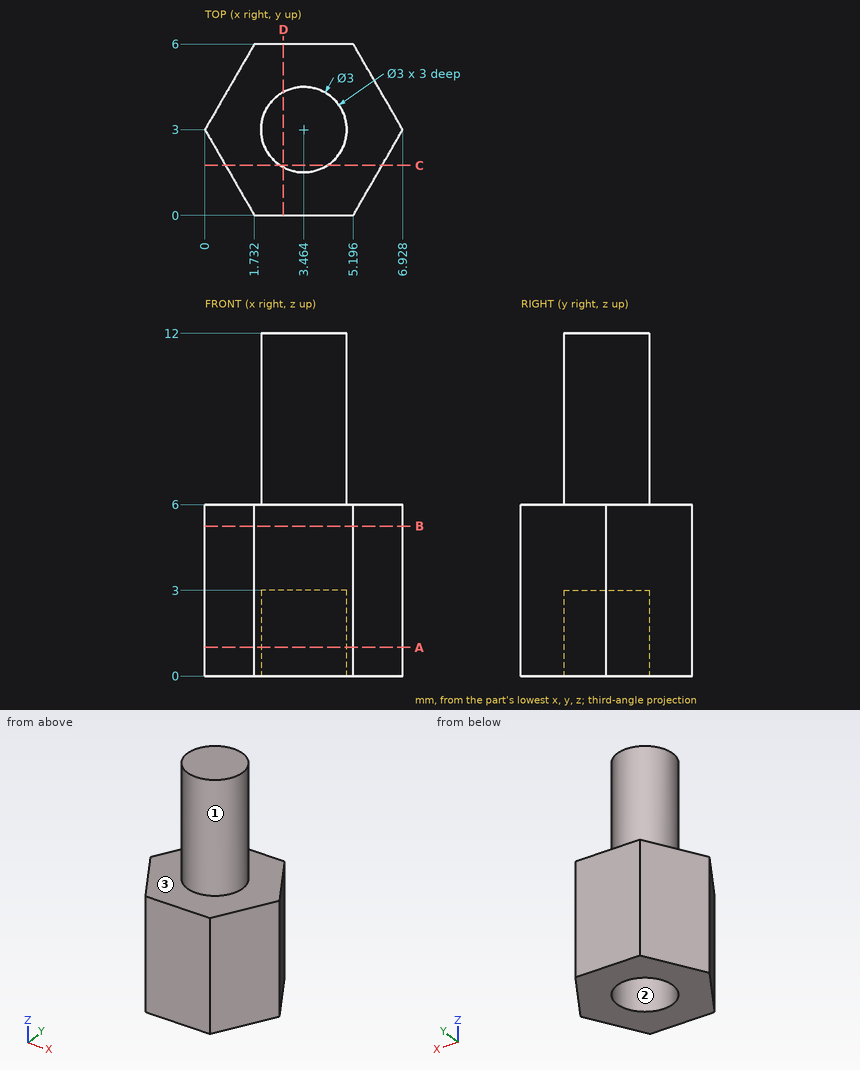
Part print with two shaded views. Sizes in mm from the minimum x, y, z corner. Round coordinates to 2 decimals unless told otherwise and drop trailing zeros. Loops run counter-clockwise (first coordinate to the right, second up) from the corner with the lowest first, then second, coordinate; pieces in that order, holes last.
1. Drill centre lines: line 1 along Z through (x, y) = (3, 0.5); line 2 along Z through (x, y) = (3.5, 3); line 3 along Y through (x, z) = (2.5, 1). Where is each one in solid material? Low to high.
Solutions:
line 1: z = 0 to 6
line 2: z = 3 to 12
line 3: y = 0 to 1.85, 4.15 to 6
2. Slice it at A-A (z = 1). Give the cut face in (x, y), and give its area (3 significant figures).
Solutions:
outline: (0, 3) - (1.73, 0) - (5.2, 0) - (6.93, 3) - (5.2, 6) - (1.73, 6) - close; hole circle Ø3 at (3.46, 3)
area: 24.1 mm2
3. Slice it at D-D (x = 2.75). Give the cut face in (y, z), and give its area (3 significant figures).
Solutions:
outline: (0, 0) - (1.68, 0) - (1.68, 3) - (4.32, 3) - (4.32, 0) - (6, 0) - (6, 6) - (4.32, 6) - (4.32, 12) - (1.68, 12) - (1.68, 6) - (0, 6) - close
area: 43.9 mm2
4. Slice it at C-C (y = 1.75). Give the cut face in (x, z) (1 decimal).
Solutions:
outline: (0.7, 0) - (2.6, 0) - (2.6, 3) - (4.3, 3) - (4.3, 0) - (6.2, 0) - (6.2, 6) - (4.3, 6) - (4.3, 12) - (2.6, 12) - (2.6, 6) - (0.7, 6) - close
5. Two-plate mould, pull along X, no slides. Class the marked faces 1, 2 and 3: pulls with the +X half, pulls with the -X half, needs draft (parallel to the pull), parting line crosses it, or undercut.
Solutions:
face 1: parting line crosses it
face 2: undercut
face 3: needs draft
6. Slice it at B-B (z = 5.25). Give the cut face in (x, y), and give its area (3 significant figures).
Solutions:
outline: (0, 3) - (1.73, 0) - (5.2, 0) - (6.93, 3) - (5.2, 6) - (1.73, 6) - close
area: 31.2 mm2
7. Flat gauge pins, fed straight in: pin 1 (1.5 mm diameter, centred on y = 1, z = 6, fed in from -X); pin 2 (1.5 mm diameter, centred on x = 5.5, y = 5, fed in from -Z); pin 3 (0.9 mm diameter, centred on x = 3, y = 3.5, fed in from -Z); pin 4 (1 mm diameter, centred on y = 3, z = 7, fed in from +X). Where does each tip first touch, or does it go through?
Solutions:
pin 1: stops at x = 0.72
pin 2: stops at z = 0
pin 3: stops at z = 3
pin 4: stops at x = 4.96
